Read the model definition and answer for the solid it produces. Units are mm, in the model's axes. Face numbers are marked on the shaded views. A direction names the side the tool comes from. Give positions to 0.01 mm unless a question says otherwise; leave off trailing zeros. Order: outer loops, then holes, each group sorted by start corner. A loop starts at its lowest first (then second) coordinate and runs counter-clockwise, first axis right, second up.
```python
from build123d import *

# Parameters (mm, degrees)
BRACKET_BODY_PROFILE_R   = 20
BRACKET_BODY_PROFILE_R_2 = 8
BRACKET_BODY_32MM_DEPTH  = 16
CLEVIS_LUG_PROFILE_R     = 8
CLEVIS_LUG_18MM_DEPTH    = 18


with BuildPart() as part:
    # Bracket Body Profile → Bracket Body 32mm (new, symmetric)
    with BuildSketch(Plane.XY):
        with BuildLine():
            Line((-16, 0), (16, 0))
            Line((16, 0), (16, -48))
            Line((16, -48), (70, -48))
            Line((70, -48), (70, 8))
            ThreePointArc((70, 8), (47.647244828, 14.739708375), (38, 36))
            ThreePointArc((38, 36), (0, 74), (-38, 36))
            ThreePointArc((-38, 36), (-47.647244828, 14.739708375), (-70, 8))
            Line((-70, 8), (-70, -48))
            Line((-70, -48), (-16, -48))
            Line((-16, -48), (-16, 0))
        make_face()
        with Locations((0, 36)):
            Circle(BRACKET_BODY_PROFILE_R, mode=Mode.SUBTRACT)
        with Locations((56, -34)):
            Circle(BRACKET_BODY_PROFILE_R_2, mode=Mode.SUBTRACT)
        with Locations((56, -6)):
            Circle(BRACKET_BODY_PROFILE_R_2, mode=Mode.SUBTRACT)
        with Locations(Location((-56, -34, 0), (0, 0, 180))):
            Circle(BRACKET_BODY_PROFILE_R_2, mode=Mode.SUBTRACT)
        with Locations(Location((-56, -6, 0), (0, 0, 180))):
            Circle(BRACKET_BODY_PROFILE_R_2, mode=Mode.SUBTRACT)
    extrude(amount=BRACKET_BODY_32MM_DEPTH, both=True)

    # Clevis Lug Profile → Clevis Lug 18mm (add)
    with BuildSketch(Plane(origin=(20, 0, 0), x_dir=(0, 0, -1), z_dir=(1, 0, 0))):
        with BuildLine():
            Line((16, -48), (64, -48))
            ThreePointArc((64, -48), (79.811911333, -34.446111196), (68.834711668, -16.747932498))
            Line((68.834711668, -16.747932498), (16, 0))
            Line((16, 0), (16, -48))
        make_face()
        with Locations((64, -32)):
            Circle(CLEVIS_LUG_PROFILE_R, mode=Mode.SUBTRACT)
    clevis_lug_18mm = extrude(amount=CLEVIS_LUG_18MM_DEPTH)

    # Clevis Lug Mirror: Clevis Lug 18mm across plane
    add(clevis_lug_18mm.mirror(Plane(origin=(0, 0, 0), x_dir=(0, 0, 1), z_dir=(1, 0, 0))))


solid = part.part
```
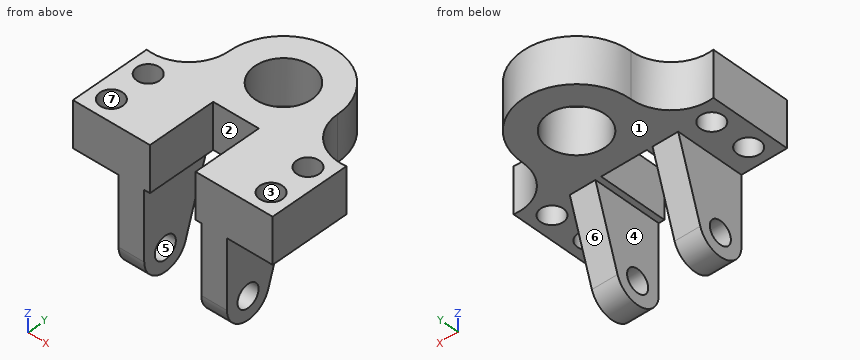
1) Given pin 1 (24 mm diameter, centred on y = -17.5, z = -39, fed in from -X); pin 2 (8 mm diameter, centred on y = -27.5, z = -44, fed in from +X); pin 3 (5 mm diameter, centred on y = 13.5, z = -6.5, fed in from +X), each flat-ended and moving along its own axis, determine where each tip first touches the part or whether it passes through.
Final values:
pin 1: stops at x = -38
pin 2: stops at x = 38
pin 3: stops at x = 53.09
2) The part is cut by section B-B on x = 0. Determine the outline of the cut face in (y, z).
Final values:
outline: (0, -16) - (16, -16) - (16, 16) - (0, 16) - close; (56, -16) - (74, -16) - (74, 16) - (56, 16) - close
3) For a pull along Z with two mould halves and no side action, classify the marked faces 5, 6 and 7 as released by +Z, released by -Z, zero draft, split by the parting line, or undercut.
Final values:
face 5: undercut
face 6: released by -Z
face 7: zero draft
4) Consider L1, parallel to Y at x = 56, z = -6; L2, parallel to X at y = -22.5, z = -51; L3, parallel to Z at x = 19, y = -34. Determine where each line is inside the solid, lowest interval first.
Final values:
L1: y = -48 to -42, -26 to -14, 2 to 9.68
L2: x = -38 to -20, 20 to 38
L3: z = -16 to 16
5) The part is cut by section D-D on y = -32. Count the separate pieces of the cut face and the enclosed holes in it, and give its area (3 significant figures).
Final values:
separate pieces: 6
enclosed holes: 0
area: 4,190 mm2
6) The part is cut by section A-A on z = -7. Determine the outline of the cut face in (x, y).
Final values:
outline: (-70, -48) - (-16, -48) - (-16, 0) - (16, 0) - (16, -48) - (70, -48) - (70, 8) arc R28.25 cw to (38, 36) arc R38 ccw to (-38, 36) arc R28.25 cw to (-70, 8) - close; hole circle Ø16 at (-56, -34); hole circle Ø16 at (-56, -6); hole circle Ø40 at (0, 36); hole circle Ø16 at (56, -34); hole circle Ø16 at (56, -6)
7) A tool of negligible diameter and unlimited length cuts with its end or side. For the marked faces 1, 2, 3 and 4, from which of +Z, -Z, +X, -X, +Y, -Y can it reach the whole face along a straight path? Write none if from no direction.
Final values:
face 1: -Z, +Y
face 2: +Z, -Z, -Y
face 3: +Z, -Z
face 4: -Z, +Y, -Y
8) The part is cut by section C-C on y = 23. Determine the outline of the cut face in (x, z), and give its area (3 significant figures).
Final values:
outline: (-41.17, -16) - (-15.2, -16) - (-15.2, 16) - (-41.17, 16) - close; (15.2, -16) - (41.17, -16) - (41.17, 16) - (15.2, 16) - close
area: 1,660 mm2
